```python
from build123d import *

# Parameters (mm, degrees)
BLOCK_BODY_260_DEPTH                   = 130
BOLT_START                             = 25
BOLT_POCKET_60X80_DEPTH                = 260
BOLT_POCKET_MIRROR_RIGHT_COPY_1_DEPTH  = 260
BOLT_HOLE_SKETCH_R                     = 10
BOLT_HOLE_CUT_DEPTH                    = 260
BOLT_HOLE_MIRROR_RIGHT_COPY_1_SKETCH_R = 10
BOLT_HOLE_MIRROR_RIGHT_COPY_1_DEPTH    = 260


with BuildPart() as part:
    # Block Profile Sketch → Block Body 260 (new, symmetric)
    with BuildSketch(Plane.XY):
        with BuildLine():
            Line((-100, 0), (-37.5, 0))
            ThreePointArc((-37.5, 0), (0, 37.5), (37.5, 0))
            Line((37.5, 0), (100, 0))
            ThreePointArc((100, 0), (0, 100), (-100, 0))
        make_face()
    extrude(amount=BLOCK_BODY_260_DEPTH, both=True)

    # Bolt Pocket Sketch → Bolt Pocket 60x80 (cut)
    with BuildSketch(Plane(origin=(0, 0, 0), x_dir=(1, 0, 0), z_dir=(0, 1, 0)).offset(BOLT_START)):
        with BuildLine():
            Line((-60, -20), (-100, -20))
            Line((-100, -20), (-100, -80))
            Line((-100, -80), (-60, -80))
            ThreePointArc((-60, -80), (-30, -50), (-60, -20))
        make_face()
    bolt_pocket_60x80 = extrude(amount=BOLT_POCKET_60X80_DEPTH, mode=Mode.SUBTRACT)

    # Bolt Pocket Mirror Front: Bolt Pocket 60x80 across plane
    add(bolt_pocket_60x80.mirror(Plane.XY), mode=Mode.SUBTRACT)

    # Bolt Pocket Mirror Right: Bolt Pocket 60x80 across plane
    add(bolt_pocket_60x80.mirror(Plane(origin=(0, 0, 0), x_dir=(0, 0, 1), z_dir=(1, 0, 0))), mode=Mode.SUBTRACT)

    # Bolt Pocket Mirror Right copy 1 sketch → Bolt Pocket Mirror Right copy 1 (cut)
    with BuildSketch(Plane(origin=(0, 0, 0), x_dir=(-1, 0, 0), z_dir=(0, 1, 0)).offset(BOLT_START)):
        with BuildLine():
            Line((-60, -20), (-100, -20))
            Line((-100, -20), (-100, -80))
            Line((-100, -80), (-60, -80))
            ThreePointArc((-60, -80), (-30, -50), (-60, -20))
        make_face()
    extrude(amount=BOLT_POCKET_MIRROR_RIGHT_COPY_1_DEPTH, mode=Mode.SUBTRACT)

    # Bolt Hole Sketch → Bolt Hole Cut (cut)
    with BuildSketch(Plane(origin=(0, 25, 0), x_dir=(1, 0, 0), z_dir=(0, 1, 0))):
        with Locations(Location((-60, -50, 0), (0, 0, 270))):
            Circle(BOLT_HOLE_SKETCH_R)
    bolt_hole_cut = extrude(amount=-BOLT_HOLE_CUT_DEPTH, mode=Mode.SUBTRACT)

    # Bolt Hole Mirror Front: Bolt Hole Cut across plane
    add(bolt_hole_cut.mirror(Plane.XY), mode=Mode.SUBTRACT)

    # Bolt Hole Mirror Right: Bolt Hole Cut across plane
    add(bolt_hole_cut.mirror(Plane(origin=(0, 0, 0), x_dir=(0, 0, 1), z_dir=(1, 0, 0))), mode=Mode.SUBTRACT)

    # Bolt Hole Mirror Right copy 1 sketch → Bolt Hole Mirror Right copy 1 (cut)
    with BuildSketch(Plane(origin=(0, 25, 0), x_dir=(-1, 0, 0), z_dir=(0, 1, 0))):
        with Locations(Location((-60, -50, 0), (0, 0, 270))):
            Circle(BOLT_HOLE_MIRROR_RIGHT_COPY_1_SKETCH_R)
    extrude(amount=-BOLT_HOLE_MIRROR_RIGHT_COPY_1_DEPTH, mode=Mode.SUBTRACT)


solid = part.part
```
The model under review builds one solid part; all positions refer to its coordinate system, in mm. A direction names the side the tool comes from. Give positions to 0.01 mm unless a question says otherwise; leave off trailing zeros. Write each loop counter-clockwise with the first axis right and the second up, starting at its lowest first coordinate (ties: lowest second). Pieces come first, ordered by that corner, then holes. Notation, with made-up numbers: (11, -18.75) -> (22, -18.75) arc R37 ccw to (22, 18.25) -> close; hole circle Ø8 at (36.5, 36.25). An arc over 180 degrees is marked (long way). Put each result on its own line as item: value.
(1) The part is to be moulded in two halves that separate along Z. For faces 1 (the flat face through (-1, 51, 130)), 2 (the flat face through (-74, 46, 20)), 3 (the flat face through (68, 0, 2)), say which applies: pulls with the +Z half, pulls with the -Z half, needs draft (parallel to the pull), parting line crosses it, or undercut.
Results are:
face 1: pulls with the +Z half
face 2: undercut
face 3: needs draft
(2) For pin 1 Ø5 at (x, z) = (22, 87.5) entering from +Y; pin 2 Ø10 at (x, y) = (-8.5, 26.5) entering from -Z; pin 3 Ø1 at (y, z) = (32, -83.5) entering from -X; pin 4 Ø4 at (y, z) = (17.5, 53.5) entering from -X, all flat-tipped, find the tip position at first contact; note any pin that passes through.
Results are:
pin 1: y = 98.08
pin 2: through
pin 3: x = -94.91
pin 4: x = -98.79
(3) We need section B-B, the plane z = 50. Give the boundary of the cut face in (x, y).
Results are:
outline: (-100, 0) -> (-70, 0) -> (-70, 25) -> (-96.82, 25) arc R100 ccw to start; (-50, 0) -> (-37.5, 0) arc R37.5 cw to (37.5, 0) -> (50, 0) -> (50, 25) -> (30, 25) -> (30, 95.39) arc R100 ccw to (-30, 95.39) -> (-30, 25) -> (-50, 25) -> close; (70, 0) -> (100, 0) arc R100 ccw to (96.82, 25) -> (70, 25) -> close
(4) We need section A-A, the plane y = 20.5. Give the boundary of the cut face in (x, z), and give its area (3 significant figures).
Results are:
outline: (-97.88, -130) -> (-31.4, -130) -> (-31.4, 130) -> (-97.88, 130) -> close; (31.4, -130) -> (97.88, -130) -> (97.88, 130) -> (31.4, 130) -> close; hole circle Ø20 at (-60, -50); hole circle Ø20 at (-60, 50); hole circle Ø20 at (60, -50); hole circle Ø20 at (60, 50)
area: 33,300 mm²
(5) To check wall thickness, follow probe 1 along Z at (x, y) = (74.5, 29); probe 2 along Z at (x, y) = (60, 6.25); probe 3 along X at (y, z) = (22.5, 43.5). State the ranges of each line that lie inside material, in increasing order. Write a range as from..to.
Results are:
probe 1: -130..-80, -20..20, 80..130
probe 2: -130..-60, -40..40, 60..130
probe 3: -97.44..-67.6, -52.4..-30, 30..52.4, 67.6..97.44
(6) We need section C-C, the plane y = 43. Give the boundary of the cut face in (x, z).
Results are:
outline: (-90.28, -130) -> (90.28, -130) -> (90.28, -80) -> (60, -80) arc R30 cw to (60, -20) -> (90.28, -20) -> (90.28, 20) -> (60, 20) arc R30 cw to (60, 80) -> (90.28, 80) -> (90.28, 130) -> (-90.28, 130) -> (-90.28, 80) -> (-60, 80) arc R30 cw to (-60, 20) -> (-90.28, 20) -> (-90.28, -20) -> (-60, -20) arc R30 cw to (-60, -80) -> (-90.28, -80) -> close
(7) Tool access review of faces 4 (the flat face through (71, 25, 50)), 5 (the flat face through (-71, 25, 50)), 6 (the cylindrical face through (-60, 13, 40)): name each direction out of +Z, -Z, +X, -X, +Y, -Y from which nothing blocks a thin tool from reaching the whole face with its end or side.
Results are:
face 4: +X, +Y
face 5: -X, +Y
face 6: +Y, -Y
(8) We need section D-D, the plane x = 42. Give the boundary of the cut face in (y, z).
Results are:
outline: (0, -130) -> (90.75, -130) -> (90.75, -74) -> (25, -74) -> (25, -26) -> (90.75, -26) -> (90.75, 26) -> (25, 26) -> (25, 74) -> (90.75, 74) -> (90.75, 130) -> (0, 130) -> close
